Drawing for the job (mm, zero at the part's lowest x, y, z). A direction names the side the tool comes from. Round coordinates to 2 decimals unless told otherwise and drop trailing zeros. Order: outer loops, then holes, each group sorted by start corner. A loop starts at its lowest first (then second) coordinate and runs counter-clockwise, first axis right, second up. Notation, with made-up numbers: (-16, 26) - (-3, 26) arc R12 cw to (-3, 48) - close; hole circle Ø8 at (36.5, -40). An arc over 180 degrees is marked (long way). One line per question, with ' | ' between items. Start each with the question number.
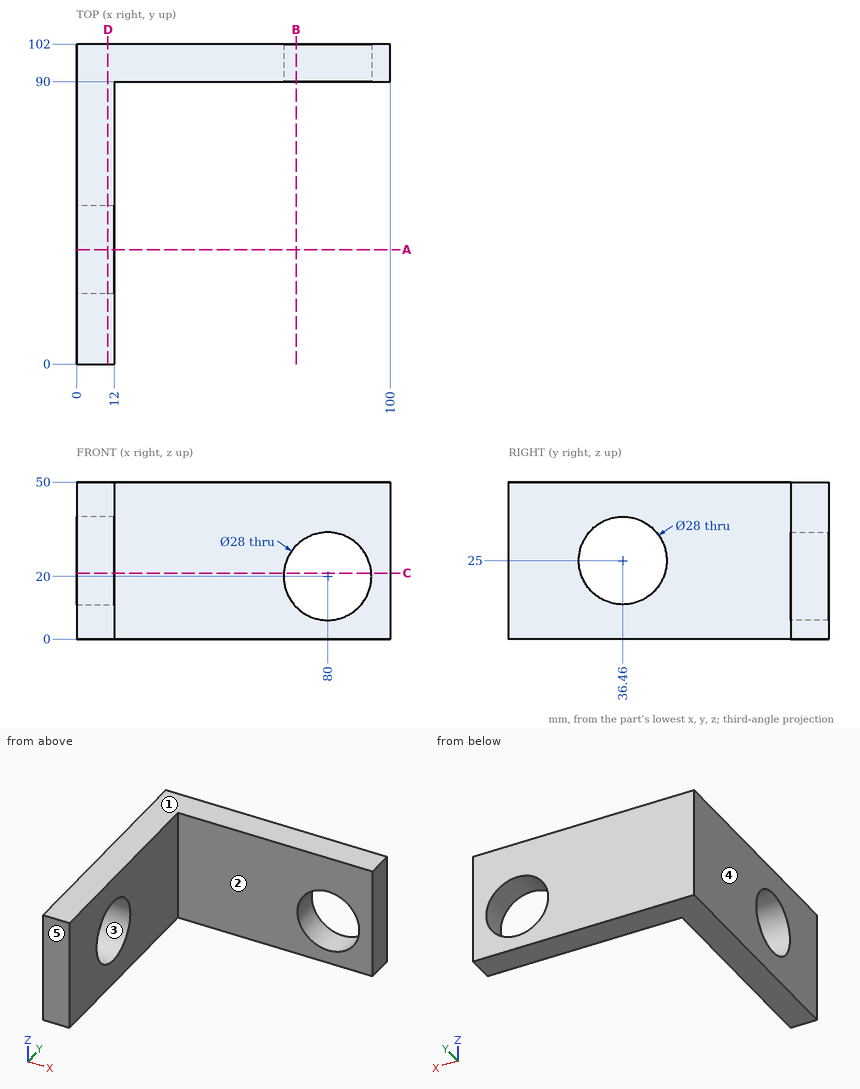
Item 1: Slice it at D-D (x = 10). Write the cut outline in (y, z).
Item 2: 3-axis set-ups, long thin cutter, end or side, ignore diameter. For the marked faces 1 and 2: which of +Z, -Z, +X, -X, +Y, -Y reach the whole face in a straight line?
Item 3: Wall check: line 1 along Z through (x, y) = (7.25, 36.46); line 2 along Z through (x, y) = (80, 98); line 3 along Y through (x, z) = (8, 25). Give the ranges that are in metal, low to high. Write a range as [from, to].
Item 4: Pin check, flat tips, straight feed: pin 1 (6 mm diameter, centred on y = 39, z = 39.5, fed in from +X); pin 2 (25 mm diameter, centred on x = 54.5, z = 23.5, fed in from -Y). Stop position of each tip, or through.
Item 5: Pull direction Y, two halves, no side cores. Call the marked faces 3, 4 and 5: released by +Y, released by -Y, zero draft, split by the parting line, or undercut.
Item 6: Slice it at B-B (x = 70). Write the cut outline in (y, z).
Item 7: Slice it at C-C (z = 21). Write the cut outline in (x, y).
Item 8: Slice it at A-A (y = 36.46). Write the cut outline in (x, z).
A:
1) outline: (0, 0) - (102, 0) - (102, 50) - (0, 50) - close; hole circle Ø28 at (36.46, 25)
2) face 1: +Z, +X, -X, +Y, -Y | face 2: +Z, -Z, +X, -Y
3) line 1: [0, 11], [39, 50] | line 2: [0, 6], [34, 50] | line 3: [0, 22.46], [50.46, 102]
4) pin 1: x = 12 | pin 2: y = 90
5) face 3: undercut | face 4: zero draft | face 5: released by -Y
6) outline: (90, 0) - (102, 0) - (102, 10.2) - (90, 10.2) - close; (90, 29.8) - (102, 29.8) - (102, 50) - (90, 50) - close
7) outline: (0, 0) - (12, 0) - (12, 23.04) - (0, 23.04) - close; (0, 49.88) - (12, 49.88) - (12, 90) - (66.04, 90) - (66.04, 102) - (0, 102) - close; (93.96, 90) - (100, 90) - (100, 102) - (93.96, 102) - close
8) outline: (0, 0) - (12, 0) - (12, 11) - (0, 11) - close; (0, 39) - (12, 39) - (12, 50) - (0, 50) - close
